from build123d import *
from build123d.topology import SkipClean

# Parameters (mm, degrees)
BASE_PLATE_SKETCH_W            = 20
BASE_PLATE_SKETCH_H            = 66
BASE_PLATE_DEPTH               = 120
UPRIGHT_WEB_SKETCH_R           = 22
UPRIGHT_WEB_SKETCH_R_2         = 11
UPRIGHT_WEB_DEPTH              = 10
TRUNNION_BOSS_FRONT_SKETCH_R   = 22
TRUNNION_BOSS_FRONT_SKETCH_R_2 = 11
TRUNNION_BOSS_FRONT_DEPTH      = 20
TRUNNION_START                 = 10
TRUNNION_BOSS_REAR_SKETCH_R    = 22
TRUNNION_BOSS_REAR_SKETCH_R_2  = 11
TRUNNION_BOSS_REAR_DEPTH       = 10
BRACKET_HOLES_SKETCH_R         = 7.5
BRACKET_HOLES_DEPTH            = 30
SEMI_CIRCULAR_BASE_DEPTH       = 64
GUSSET_1_DEPTH                 = 5
GUSSET_START                   = -64
GUSSET_2_DEPTH                 = 64
TRUNNION_START_2               = 0.5
TRUNNION_FACE_PAD_SKETCH_R     = 22
TRUNNION_FACE_PAD_SKETCH_R_2   = 11
TRUNNION_FACE_PAD_0_5MM_DEPTH  = 0.5
BASE_MOUNTING_LUGS_SKETCH_R    = 6
BASE_MOUNTING_LUGS_DEPTH       = 22


with BuildPart() as part:
    # Base Plate Sketch → Base Plate (new body)
    with BuildSketch(Plane.XY):
        Rectangle(BASE_PLATE_SKETCH_W, BASE_PLATE_SKETCH_H)
    extrude(amount=BASE_PLATE_DEPTH)

    # Upright Web Sketch → Upright Web (add)
    # profile 1 of 2: a face of its own
    with BuildSketch(Plane(origin=(10, 0, 0), x_dir=(0, 0, -1), z_dir=(1, 0, 0))):
        with BuildLine():
            Line((-76.38555148, 81.680384964), (-120, 33))
            Line((-120, 33), (0, 33))
            Line((0, 33), (-43.61444852, 81.680384964))
            ThreePointArc((-43.61444852, 81.680384964), (-39.451494792, 74.858685241), (-38, 67))
            ThreePointArc((-38, 67), (-67.858685241, 46.451494792), (-76.38555148, 81.680384964))
        make_face()
    # profile 2 of 2: a face of its own
    with BuildSketch(Plane(origin=(10, 0, 0), x_dir=(0, 0, -1), z_dir=(1, 0, 0))):
        with Locations((-60, 67)):
            Circle(UPRIGHT_WEB_SKETCH_R)
        with Locations(Location((-60, 67, 0), (0, 0, 90))):
            Circle(UPRIGHT_WEB_SKETCH_R_2, mode=Mode.SUBTRACT)
    extrude(amount=-UPRIGHT_WEB_DEPTH)

    # Trunnion Boss Front Sketch → Trunnion Boss Front (add)
    with SkipClean():  # the faces are left unmerged after this step: merging them gives an invalid solid
        with BuildSketch(Plane.ZY):
            with Locations(Location((60, 67, 0), (0, 0, 41.858266049))):
                Circle(TRUNNION_BOSS_FRONT_SKETCH_R)
            with Locations(Location((60, 67, 0), (0, 0, 90))):
                Circle(TRUNNION_BOSS_FRONT_SKETCH_R_2, mode=Mode.SUBTRACT)
        extrude(amount=TRUNNION_BOSS_FRONT_DEPTH)

    # Trunnion Boss Rear Sketch → Trunnion Boss Rear (add)
    with SkipClean():  # the faces are left unmerged after this step: merging them gives an invalid solid
        with BuildSketch(Plane(origin=(10, 0, 0), x_dir=(0, 0, -1), z_dir=(1, 0, 0)).offset(TRUNNION_START)):
            with Locations(Location((-60, 67, 0), (0, 0, 90))):
                Circle(TRUNNION_BOSS_REAR_SKETCH_R)
            with Locations(Location((-60, 67, 0), (0, 0, 90))):
                Circle(TRUNNION_BOSS_REAR_SKETCH_R_2, mode=Mode.SUBTRACT)
        extrude(amount=-TRUNNION_BOSS_REAR_DEPTH)

    # Bracket Holes Sketch → Bracket Holes (cut)
    with SkipClean():  # the faces are left unmerged after this step: merging them gives an invalid solid
        with BuildSketch(Plane(origin=(10, 0, 0), x_dir=(0, 0, -1), z_dir=(1, 0, 0))):
            with Locations(Location((-100, 11, 0), (0, 0, 90))):
                Circle(BRACKET_HOLES_SKETCH_R)
            with Locations(Location((-20, 11, 0), (0, 0, 90))):
                Circle(BRACKET_HOLES_SKETCH_R)
        extrude(amount=-BRACKET_HOLES_DEPTH, mode=Mode.SUBTRACT)

    # Semi-Circular Base Sketch → Semi-Circular Base (add)
    with SkipClean():  # the faces are left unmerged after this step: merging them gives an invalid solid
        with BuildSketch(Plane(origin=(10, 0, 0), x_dir=(0, 0, -1), z_dir=(1, 0, 0))):
            with BuildLine():
                Line((-92, -33), (-78, -33))
                ThreePointArc((-78, -33), (-60, -15), (-42, -33))
                Line((-42, -33), (-28, -33))
                ThreePointArc((-28, -33), (-60, -1), (-92, -33))
            make_face()
        extrude(amount=SEMI_CIRCULAR_BASE_DEPTH)



with BuildPart() as body_2:
    # Gusset 1 Sketch → Gusset 1 (new, symmetric)
    with BuildSketch(Plane.XY.offset(60)):
        Polygon((10, -5), (10, 46.478793063), (20, 46.478793063), (74, -1), (74, -5), align=None)
    extrude(amount=GUSSET_1_DEPTH, both=True)


with BuildPart() as part_1:
    with SkipClean():  # the faces are left unmerged after this step: merging them gives an invalid solid
        add(part.part)

        add(body_2.part)  # Gusset 2 merges body 2
        # Gusset 2 Sketch → Gusset 2 (add)
        with BuildSketch(Plane(origin=(74, 0, 0), x_dir=(0, 0, -1), z_dir=(1, 0, 0)).offset(GUSSET_START)):
            with BuildLine():
                Line((-92, -33), (-78, -33))
                ThreePointArc((-78, -33), (-60, -15), (-42, -33))
                Line((-42, -33), (-28, -33))
                ThreePointArc((-28, -33), (-60, -1), (-92, -33))
            make_face()
        extrude(amount=GUSSET_2_DEPTH)

    # Trunnion Face Pad Sketch → Trunnion Face Pad 0.5mm (add)
    with SkipClean():  # the faces are left unmerged after this step: merging them gives an invalid solid
        with BuildSketch(Plane(origin=(20, 0, 0), x_dir=(0, 0, -1), z_dir=(1, 0, 0)).offset(TRUNNION_START_2)):
            with Locations(Location((-60, 67, 0), (0, 0, 138.141733951))):
                Circle(TRUNNION_FACE_PAD_SKETCH_R)
            with Locations(Location((-60, 67, 0), (0, 0, 90))):
                Circle(TRUNNION_FACE_PAD_SKETCH_R_2, mode=Mode.SUBTRACT)
        extrude(amount=-TRUNNION_FACE_PAD_0_5MM_DEPTH)

    # Base Mounting Lugs Sketch → Base Mounting Lugs (add)
    # profile 1 of 2: a face of its own
    with SkipClean():  # the faces are left unmerged after this step: merging them gives an invalid solid
        with BuildSketch(Plane.XZ.offset(33)):
            with BuildLine():
                Line((27, 100), (27, 83))
                Line((27, 83), (57, 83))
                Line((57, 83), (57, 85))
                Line((57, 85), (57, 100))
                ThreePointArc((57, 100), (42, 115), (27, 100))
            make_face()
            with Locations(Location((42, 100, 0), (0, 0, 270))):
                Circle(BASE_MOUNTING_LUGS_SKETCH_R, mode=Mode.SUBTRACT)
        # profile 2 of 2: a face of its own
        with BuildSketch(Plane.XZ.offset(33)):
            with BuildLine():
                Line((27, 20), (27, 38))
                Line((27, 38), (57, 38))
                Line((57, 38), (57, 35))
                Line((57, 35), (57, 20))
                ThreePointArc((57, 20), (42, 5), (27, 20))
            make_face()
            with Locations(Location((42, 20, 0), (0, 0, 270))):
                Circle(BASE_MOUNTING_LUGS_SKETCH_R, mode=Mode.SUBTRACT)
        extrude(amount=-BASE_MOUNTING_LUGS_DEPTH)


solid = part_1.part
Geometry: final body of the model. Coordinates: model frame, mm. A direction names the side the tool comes from. Coordinates: 2 decimals unless noted, no trailing zeros. Order: outer loops, then holes, each group sorted by start corner. A loop starts at its lowest first (then second) coordinate and runs counter-clockwise, first axis right, second up.
(1) Section query A-A (z = 60). Return the cut outline in (x, y).
(2) Section query C-C (x = 42). Return the cut outline in (y, z).
(3) Section query D-D (y = 11). Return the cut outline in (x, z), plus the area to 3 significant figures.
(4) Material intervals for probe 1 along Z at (x, y) = (-3, 11); probe 2 along X at (y, z) = (-21, 20); probe 3 along X at (y, z) = (17.5, 89), sorted ascending.
(5) First-contact query: pin 1 (1 mm diameter, centred on y = -5, z = 23, fed in from +X); pin 2 (5 mm diameter, centred on x = -3.5, z = 70, fed in from +Y); pin 3 (5 mm diameter, centred on y = -19.5, z = 30, fed in from -X). Flat tips, straight axial feed; report the tip coordinate or a pass-through.
(6) Draft query along Z for faces 5 (the face through (42, -15, 60)), 6 (the face through (74, -13, 60)), 7 (the face through (35, 17, 55)), 8 (the face through (35, 17, 65)). Return one class per face: pulls with the +Z half, pulls with the -Z half, needs draft (parallel to the pull), parting line crosses it, or undercut.
(7) Section query B-B (y = 59). Return the cut outline in (x, z), plus the area to 3 significant figures.
(8) Access query for faces 1 (the face through (-5, 33, 59)), 2 (the face through (42, -11, 28)), 3 (the face through (10, -26, 60)), 4 (the face through (27, -20, 25)). Directions: +Z, -Z, +X, -X, +Y, -Y. A direction counts if a zero-diameter tool reaches every point of the face in a straight line with its end or side. Return the directions, or none.
Solution:
1. outline: (-20, 45) - (0, 45) - (0, 33) - (-10, 33) - (-10, -33) - (10, -33) - (10, -15) - (74, -15) - (74, -1) - (20.5, 46.04) - (20.5, 56) - (-20, 56) - close; (-20, 78) - (20.5, 78) - (20.5, 89) - (-20, 89) - close
2. outline: (-33, 5) - (-11, 5) - (-11, 14) - (-33, 14) - close; (-33, 26) - (-11, 26) - (-11, 36.76) arc R32 ccw to (-1.39, 55) - (27.14, 55) - (27.14, 65) - (-1.39, 65) arc R32 ccw to (-11, 83.24) - (-11, 94) - (-33, 94) - (-33, 78) arc R18 cw to (-33, 42) - close; (-33, 106) - (-11, 106) - (-11, 115) - (-33, 115) - close
3. outline: (-10, 0) - (10, 0) - (10, 12.5) - (-10, 12.5) - close; (-10, 27.5) - (10, 27.5) - (10, 55) - (60.35, 55) - (60.35, 65) - (10, 65) - (10, 92.5) - (-10, 92.5) - close; (-10, 107.5) - (10, 107.5) - (10, 120) - (-10, 120) - close
3. area: 2,300 mm2
4. probe 1: z = 0 to 12.5, 27.5 to 92.5, 107.5 to 120
4. probe 2: x = -10 to 10, 27 to 36, 48 to 57
4. probe 3: x = -10 to 10
5. pin 1: stops at x = 10
5. pin 2: stops at y = 87.68
5. pin 3: stops at x = -10
6. face 5: undercut
6. face 6: needs draft
6. face 7: pulls with the -Z half
6. face 8: pulls with the +Z half
7. outline: (-20, 39.51) - (0, 39.51) - (0, 23.29) - (10, 23.29) - (10, 39.51) - (20.5, 39.51) - (20.5, 52.45) - (-20, 52.45) - close; (-20, 67.55) - (20.5, 67.55) - (20.5, 80.49) - (10, 80.49) - (10, 96.71) - (0, 96.71) - (0, 80.49) - (-20, 80.49) - close
7. area: 1,370 mm2
8. face 1: +Z, -Z, -X
8. face 2: -Z, +X, +Y
8. face 3: +X, -Y
8. face 4: -Z, +Y
